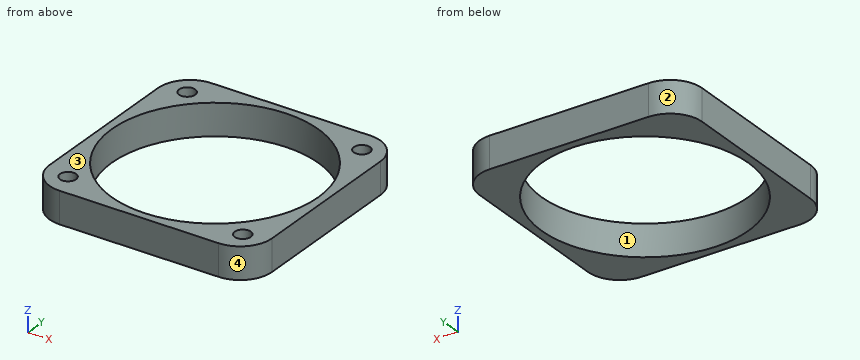
from build123d import *

# Parameters (mm, degrees)
SKETCH1_R              = 65
BOSS_EXTRUDE1_DEPTH    = 20
M12_TAPPED_HOLE1_D     = 10.2
M12_TAPPED_HOLE1_DEPTH = 16
M12_TAPPED_HOLE1_TIP   = 3.064389157


with BuildPart() as part:
    # Sketch1 → Boss-Extrude1 (new body)
    with BuildSketch(Plane.XY):
        with BuildLine():
            Line((20, 0), (120, 0))
            ThreePointArc((120, 0), (134.142135624, 5.857864376), (140, 20))
            Line((140, 20), (140, 120))
            ThreePointArc((140, 120), (134.142135624, 134.142135624), (120, 140))
            Line((120, 140), (20, 140))
            ThreePointArc((20, 140), (5.857864376, 134.142135624), (0, 120))
            Line((0, 120), (0, 20))
            ThreePointArc((0, 20), (5.857864376, 5.857864376), (20, 0))
        make_face()
        with Locations((70, 70)):
            Circle(SKETCH1_R, mode=Mode.SUBTRACT)
    extrude(amount=BOSS_EXTRUDE1_DEPTH)

    # M12 Tapped Hole1
    with Locations(Plane(origin=(15, 125, 20), x_dir=(1, 0, 0), z_dir=(0, 0, 1))):
        with Locations((0, 0), (110, 0), (110, -110), (0, -110)):
            Hole(M12_TAPPED_HOLE1_D / 2, depth=M12_TAPPED_HOLE1_DEPTH)
            with Locations((0, 0, -(M12_TAPPED_HOLE1_DEPTH + M12_TAPPED_HOLE1_TIP / 2))):  # 118° drill point
                Cone(0, M12_TAPPED_HOLE1_D / 2, M12_TAPPED_HOLE1_TIP, mode=Mode.SUBTRACT)


solid = part.part
Model file for the job. Use its own axes, mm. Face numbers are marked on the shaded views. Coordinates: 2 decimals unless noted, no trailing zeros. Write each loop counter-clockwise with the first axis right and the second up, starting at its lowest first coordinate (ties: lowest second). Pieces come first, ordered by that corner, then holes. Notation, with made-up numbers: (69, -33) - (128, -33) arc R22 ccw to (128, -26) - close; hole circle Ø1 at (11, 6.5). An arc over 180 degrees is marked (long way). Write each question's results on one line, items separated by ' | '. Start each with the question number.
1) Cut at A-A (y = 70). Write the cut outline in (x, z), then the cut area to 3 significant figures.
2) Probe line 1 along X through (y, z) = (15, 14.75); line 2 along Y through (x, z) = (85, 3.75). List the from-to ranges inside material, lowest first. Write a range as from..to.
3) Mould opens along X. For the marked faces 1, 2, 3 and 4 say: pulls with the +X half, pulls with the -X half, needs draft (parallel to the pull), parting line crosses it, or undercut.
4) Cut at B-B (x = 107). Write the cut outline in (y, z), then the cut area to 3 significant figures.
Returned:
1) outline: (0, 0) - (5, 0) - (5, 20) - (0, 20) - close; (135, 0) - (140, 0) - (140, 20) - (135, 20) - close | area: 200 mm^2
2) line 1: 0.64..9.9, 20.1..35.36, 104.64..119.9, 130.1..139.36 | line 2: 0..6.75, 133.25..140
3) face 1: undercut | face 2: pulls with the -X half | face 3: needs draft | face 4: pulls with the +X half
4) outline: (0, 0) - (16.56, 0) - (16.56, 20) - (0, 20) - close; (123.44, 0) - (140, 0) - (140, 20) - (123.44, 20) - close | area: 662 mm^2
